The listing builds one solid part. Answer for the finished solid, in the listing's coordinates (mm). Coordinates: 2 decimals unless noted, no trailing zeros. Order: outer loops, then holes, each group sorted by start corner. A loop starts at its lowest first (then second) coordinate and runs counter-clockwise, first axis right, second up. Notation, with made-up numbers: (47, 16.25) -> (74, 16.25) arc R22 cw to (74, 49.25) -> close; hole circle Ø2 at (32, 44). An arc over 180 degrees is marked (long way). Write each question's results on one line, items separated by ' | '. Start each with the question number.
(1) The part is cut by section C-C, the plane z = 162. Give the vertices of the cut face in (x, y).
(2) Given pin 1 (3 mm diameter, centred on y = 2, z = 197, fed in from +X); pin 2 (4 mm diameter, centred on x = 5, z = 212.5, fed in from -Y); pin 3 (2 mm diameter, centred on x = -0.5, y = 6.5, fed in from +Z), each flat-ended and moving along its own axis, determine where each tip first touches the part or whether it passes through.
(3) The part is cut by section A-A, the plane y = 0. Give the vertices of the cut face in (x, z).
(4) Straight lines are drawn through the part: L1, parallel to Z at x = 4.5, y = 4.5; L2, parallel to X at y = 0, z = 199; L3, parallel to Y at x = 0.25, z = 146.5. For each, find the intervals that lie inside material, in ascending order.
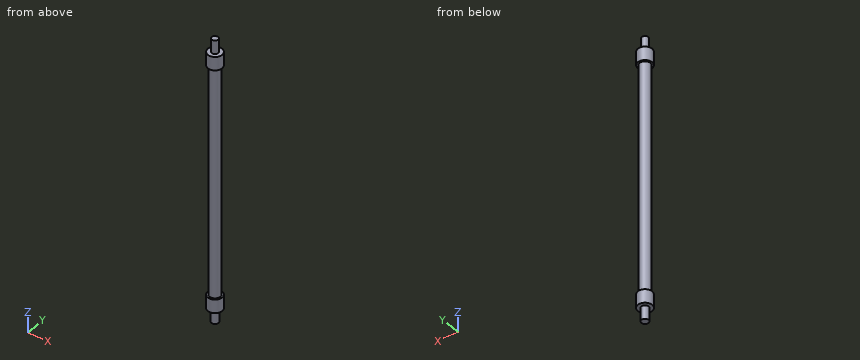
```python
from build123d import *

# Parameters (mm, degrees)
SKETCH_1_R      = 4
EXTRUDE_1_DEPTH = 15
SKETCH_2_R      = 6
EXTRUDE_2_DEPTH = 270
SKETCH_3_R      = 8
EXTRUDE_3_DEPTH = 15
SKETCH_4_R      = 8
EXTRUDE_4_DEPTH = 15
SKETCH_5_R      = 3.5
EXTRUDE_5_DEPTH = 15


with BuildPart() as part:
    # 草图1 → 凸台-拉伸1 (new body)
    with BuildSketch(Plane.XY):
        Circle(SKETCH_1_R)
    extrude(amount=EXTRUDE_1_DEPTH)

    # 草图2 → 凸台-拉伸2 (add)
    with BuildSketch(Plane.XY.offset(15)):
        Circle(SKETCH_2_R)
    extrude(amount=EXTRUDE_2_DEPTH)

    # 草图3 → 凸台-拉伸3 (add)
    with BuildSketch(Plane(origin=(0, 0, 15), x_dir=(-1, 0, 0), z_dir=(0, 0, -1))):
        Circle(SKETCH_3_R)
    extrude(amount=-EXTRUDE_3_DEPTH)

    # 草图4 → 凸台-拉伸4 (add)
    with BuildSketch(Plane.XY.offset(285)):
        with Locations(Location((0, 0, 0), (0, 0, 180))):
            Circle(SKETCH_4_R)
    extrude(amount=EXTRUDE_4_DEPTH)

    # 草图5 → 凸台-拉伸5 (add)
    with BuildSketch(Plane.XY.offset(300)):
        Circle(SKETCH_5_R)
    extrude(amount=EXTRUDE_5_DEPTH)


solid = part.part
```
Established:
1) outline: circle Ø12 at (0, 0)
2) pin 1: stops at x = 5.98 | pin 2: stops at y = -5.2 | pin 3: stops at z = 300
3) outline: (-8, 15) -> (-4, 15) -> (-4, 0) -> (4, 0) -> (4, 15) -> (8, 15) -> (8, 30) -> (6, 30) -> (6, 285) -> (8, 285) -> (8, 300) -> (3.5, 300) -> (3.5, 315) -> (-3.5, 315) -> (-3.5, 300) -> (-8, 300) -> (-8, 285) -> (-6, 285) -> (-6, 30) -> (-8, 30) -> close
4) L1: z = 15 to 30, 285 to 300 | L2: x = -6 to 6 | L3: y = -5.99 to 5.99
